```python
from build123d import *

# Parameters (mm, degrees)
EXTRUDE_1_DEPTH       = 20
HOLE_WIZARD_9_0_9_1_D = 9
HOLE_WIZARD_M6_1_D    = 5
FILLET_1_R            = 10
CHAMFER_1_SIZE        = 2
HOLE_WIZARD_M4_1_D    = 3.3


with BuildPart() as part:
    # 草图1 → 凸台-拉伸1 (new body)
    with BuildSketch(Plane.XY):
        Polygon((15, 310), (-15, 310), (-15, 20), (-32.5, 20), (-32.5, 0), (32.5, 0), (32.5, 20), (15, 20), align=None)
    extrude(amount=EXTRUDE_1_DEPTH)

    # Ø9.0 (9) 直径孔1 (through all)
    with Locations(Plane(origin=(0, 20, 0), x_dir=(1, 0, 0), z_dir=(0, 1, 0))):
        with Locations((22.5, -10), (-22.5, -10)):
            Hole(HOLE_WIZARD_9_0_9_1_D / 2)

    # M6 螺纹孔1 (through all)
    with Locations(Plane.XY.offset(20)):
        with Locations((0, 280), (0, 150), (0, 20), (0, 260), (0, 140)):
            Hole(HOLE_WIZARD_M6_1_D / 2)

    # 圆角1
    fillet_1_edges = [part.edges().sort_by_distance(p)[0] for p in [
        (0, 310, 0),
    ]]
    fillet(fillet_1_edges, radius=FILLET_1_R)

    # 倒角1
    chamfer_1_edges = [part.edges().sort_by_distance(p)[0] for p in [
        (-32.5, 10, 20),
        (32.5, 10, 20),
        (32.5, 10, 0),
        (-32.5, 10, 0),
    ]]
    chamfer(chamfer_1_edges, length=CHAMFER_1_SIZE)

    # M4 螺纹孔1 (through all)
    with Locations(Plane.ZY.offset(15)):
        with Locations((6, 285), (6, 270)):
            Hole(HOLE_WIZARD_M4_1_D / 2)


solid = part.part
```
Geometry: final body of the model. Coordinates: model frame, mm. A direction names the side the tool comes from. Give positions to 0.01 mm unless a question says otherwise; leave off trailing zeros. Loops run counter-clockwise (first coordinate to the right, second up) from the corner with the lowest first, then second, coordinate; pieces in that order, holes last. Notation, with made-up numbers: (70.5, -7) -> (79.5, -7) arc R26 cw to (79.5, 25) -> close; hole circle Ø6 at (83, -5). An arc over 180 degrees is marked (long way). Use CSV: the item, a comma, the result in double quotes.
(1) Ray query, line 1 along Y through (x, z) = (0, 9.5); line 2 along X through (y, z) = (150, 7.25); line 3 along Y through (x, z) = (5.5, 6.75). Return the intervals inside material, ascending. Write a range as [from, to].
From the geometry:
line 1,"[0, 17.5], [22.5, 137.5], [142.5, 147.5], [152.5, 257.5], [262.5, 277.5], [282.5, 309.99]"
line 2,"[-15, -2.5], [2.5, 15]"
line 3,"[0, 268.53], [271.47, 283.53], [286.47, 309.46]"
(2) Access query for faces 4 (the face through (15, 163, 10)), 5 (the face through (-28, 20, 10)), 6 (the face through (0, 310, 15)). Directions: +Z, -Z, +X, -X, +Y, -Y. A direction counts if a zero-diameter tool reaches every point of the face in a straight line with its end or side. Return the directions, or none.
From the geometry:
face 4,"+Z, -Z, +X, +Y"
face 5,"+Z, -Z, -X, +Y"
face 6,"+Z, -Z, +X, -X, +Y"
(3) Cut plane B-B (y = 50). Output: boundary loops of the cut face in (x, z), plus the area to 3 significant figures.
From the geometry:
outline,"(-15, 0) -> (15, 0) -> (15, 20) -> (-15, 20) -> close"
area,"600 mm^2"
(4) First-contact query: P1, Ø6, axis at x = 0, y = 20, coming from the -Z side; P2, Ø10, axis at y = 269.5, z = 15, coming from the -X side; P3, Ø8, axis at y = 54.5, z = 8.5, coming from the +X side; P4, Ø9, axis at x = 21, z = 12.5, coming from the +Y side. Flat tips, straight axial feed; report the tip coordinate or a pass-through.
From the geometry:
P1,"z = 0"
P2,"x = -15"
P3,"x = 15"
P4,"y = 20"
(5) Cut plane A-A (x = 24). Output: boundary loops of the cut face in (y, z).
From the geometry:
outline,"(0, 0) -> (20, 0) -> (20, 5.76) -> (0, 5.76) -> close; (0, 14.24) -> (20, 14.24) -> (20, 20) -> (0, 20) -> close"
(6) Pull-direction query (X, two-part tool) for faces 1 (the face through (28, 20, 10)), 2 (the face through (32.5, 10, 10)), 3 (the face through (27, 10, 10)); classes: released by +X, released by -X, zero draft, split by the parting line, or undercut.
From the geometry:
face 1,"zero draft"
face 2,"released by +X"
face 3,"undercut"
